Can you work these out from the model? Positions are in its coordinate system, mm. Face numbers are marked on the shaded views. A direction names the side the tool comes from. Give positions to 0.01 mm unless a question says otherwise; leave off trailing zeros. Order: outer loops, then holes, each group sorted by start corner. A loop starts at its lowest first (then second) coordinate and runs counter-clockwise, first axis right, second up.
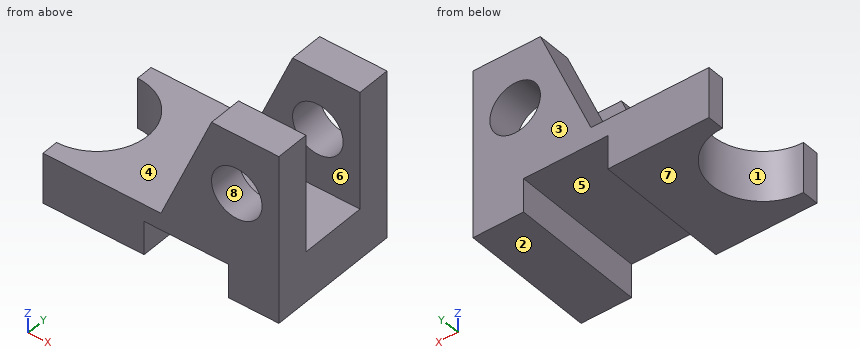
```python
from build123d import *

# Parameters (mm, degrees)
BASE_BLOCK_DEPTH           = 30
SIDE_BOSS_DEPTH            = 20
TOP_BOSS_DEPTH             = 20
THROUGH_HOLE_SKETCH_R      = 15
COAXIAL_THROUGH_HOLE_DEPTH = 80
CURVED_RELIEF_SKETCH_W     = 50
CURVED_RELIEF_SKETCH_H     = 20
CURVED_RELIEF_CUT_DEPTH    = 80


with BuildPart() as part:
    # Base Profile Sketch → Base Block (new body)
    with BuildSketch(Plane.XY):
        with BuildLine():
            Line((140, 0), (0, 0))
            Line((0, 0), (0, -10))
            ThreePointArc((0, -10), (30, -40), (0, -70))
            Line((0, -70), (0, -80))
            Line((0, -80), (140, -80))
            Line((140, -80), (140, 0))
        make_face()
    extrude(amount=BASE_BLOCK_DEPTH)

    # Side Boss Sketch → Side Boss (add)
    with BuildSketch(Plane.XZ.offset(80)):
        Polygon((140, 30), (140, 100), (100, 100), (70, 30), align=None)
    extrude(amount=-SIDE_BOSS_DEPTH)

    # Top Boss Sketch → Top Boss (add)
    with BuildSketch(Plane(origin=(0, 0, 0), x_dir=(1, 0, 0), z_dir=(0, 1, 0))):
        Polygon((140, -30), (140, -100), (100, -100), (70, -30), align=None)
    extrude(amount=-TOP_BOSS_DEPTH)

    # Through Hole Sketch → Coaxial Through Hole (cut)
    with BuildSketch(Plane.XZ.offset(80)):
        with Locations(Location((115, 65, 0), (0, 0, 270))):
            Circle(THROUGH_HOLE_SKETCH_R)
    extrude(amount=-COAXIAL_THROUGH_HOLE_DEPTH, mode=Mode.SUBTRACT)

    # Curved Relief Sketch → Curved Relief Cut (cut)
    with BuildSketch(Plane.XZ.offset(80)):
        with Locations((85, 10)):
            Rectangle(CURVED_RELIEF_SKETCH_W, CURVED_RELIEF_SKETCH_H)
    extrude(amount=-CURVED_RELIEF_CUT_DEPTH, mode=Mode.SUBTRACT)


solid = part.part
```
1) Suppose I cut it at D-D (x = 16). Please give me the cut outline in (y, z).
2) Suppose I cut it at B-B (z = 65). Please give me the cut outline in (x, y), and give its area (3 significant figures).
3) I'm going to push flat-ended pins straight in: pin 1 Ø6 at (x, z) = (88, 14.5) entering from +Y; pin 2 Ø10 at (x, y) = (21, -66.5) entering from +Z; pin 3 Ø10 at (y, z) = (-33.5, 5) entering from -X; pin 4 Ø8 at (x, y) = (70.5, -71.5) entering from +Z. Where does each tip first touch, or does it pass through?
4) Suppose I cut it at A-A (z = 9). Please give me the cut outline in (x, y).
5) If I drill on line 1 (Y direction, x = 109, z = 37.5); line 2 (Z direction, x = 59, y = -66); line 3 (X direction, y = -73, z = 60), over which ranges is the centre line in solid material (lowest first)?
6) We'd pull the mould along Y, two halves only. Please class the marked faces 1, 2 and 3: +Y half, -Y half, draft (parallel to the pull), parting line (faces both ways), or undercut.
7) Which directions (+Z, -Z, +X, -X, +Y, -Y) give clear straight access to the entire face, cutting with the end or side of a thin tool? Please do the marked faces 4, 5, 6, 7 and 8.
8) Suppose I cut it at C-C (y = -14). Please give me the cut outline in (x, z).
Results:
1. outline: (-80, 0) - (-65.38, 0) - (-65.38, 30) - (-80, 30) - close; (-14.62, 0) - (0, 0) - (0, 30) - (-14.62, 30) - close
2. outline: (85, -80) - (100, -80) - (100, -60) - (85, -60) - close; (85, -20) - (100, -20) - (100, 0) - (85, 0) - close; (130, -80) - (140, -80) - (140, -60) - (130, -60) - close; (130, -20) - (140, -20) - (140, 0) - (130, 0) - close
2. area: 1,000 mm2
3. pin 1: passes through
3. pin 2: stops at z = 30
3. pin 3: stops at x = 27.71
3. pin 4: stops at z = 40.5
4. outline: (0, -80) - (60, -80) - (60, 0) - (0, 0) - (0, -10) arc R30 cw to (0, -70) - close; (110, -80) - (140, -80) - (140, 0) - (110, 0) - close
5. line 1: y = -80 to -60, -20 to 0
5. line 2: z = 0 to 30
5. line 3: x = 82.86 to 100.86, 129.14 to 140
6. face 1: undercut
6. face 2: draft
6. face 3: +Y half
7. face 4: +Z, -X
7. face 5: -Z, +Y, -Y
7. face 6: +Z, +X, -X
7. face 7: -Z, +X, -X, +Y, -Y
7. face 8: +Y, -Y
8. outline: (14.97, 0) - (60, 0) - (60, 20) - (110, 20) - (110, 0) - (140, 0) - (140, 100) - (100, 100) - (70, 30) - (14.97, 30) - close; hole circle Ø30 at (115, 65)
